Build history of the part. All positions in model axes, mm. A direction names the side the tool comes from. Round coordinates to 2 decimals unless told otherwise and drop trailing zeros. Write each loop counter-clockwise with the first axis right and the second up, starting at its lowest first coordinate (ties: lowest second). Pieces come first, ordered by that corner, then holes.
from build123d import *

# Parameters (mm, degrees)
BOSS_EXTRUDE1_DEPTH = 6
CUT_EXTRUDE1_REACH  = 68.303
SKETCH2_R           = 4.5
CHAMFER1_SIZE       = 10


with BuildPart() as part:
    # Sketch1 → Boss-Extrude1 (new body)
    with BuildSketch(Plane.XY):
        Polygon((-33.521587555, -18.6224812), (-33.521587555, 51.3775188), (-3.521587555, 51.3775188), (-3.521587555, 23.144505274), (41.478412445, 23.144505274), (41.478412445, -18.6224812), align=None)
    extrude(amount=BOSS_EXTRUDE1_DEPTH)

    # Sketch2 → Cut-Extrude1 (cut, up to next)
    with BuildSketch(Plane.XY.offset(6), mode=Mode.PRIVATE) as cut_extrude1_sk1:
        with Locations((-18.521587555, 36.3775188)):
            Circle(SKETCH2_R)
    cut_extrude1_tool1 = extrude(cut_extrude1_sk1.sketch, amount=-CUT_EXTRUDE1_REACH, mode=Mode.PRIVATE) & part.part
    add(cut_extrude1_tool1.solids().sort_by_distance((-18.521588, 36.377519, 6))[0], mode=Mode.SUBTRACT)

    # Chamfer1
    chamfer1_edges = [part.edges().sort_by_distance(p)[0] for p in [
        (-33.521587555, -18.6224812, 3),
    ]]
    chamfer(chamfer1_edges, length=CHAMFER1_SIZE)


solid = part.part
1) Which spindle directions (+Z, -Z, +X, -X, +Y, -Y) get a long thin tool onto all of the face, cutting with end or side? Do faces 1 (the flat face through (-3.522, 37, 3)), 2 (the flat face through (-4, 9, 6)). Say none if no direction does.
Results:
face 1: +Z, -Z, +X, +Y
face 2: +Z, +X, -X, +Y, -Y
2) Mould opens along Y. For faces 3 (the flat face through (-28.452, -13.692, 2.958)), 4 (the cylindrical face through (-19.497, 31.985, 3.042)), 5 (the flat face through (-19, 51.378, 3)) say: released by +Y, released by -Y, zero draft, split by the parting line, or undercut.
Results:
face 3: released by -Y
face 4: undercut
face 5: released by +Y
3) Pin check, flat tip, straight feed: pin 1 Ø1.8 at (y, z) = (31, 1.5) entering from +X. Stop position of the tip, or through.
Results:
pin 1: stops at x = -3.52
4) Slice it at A-A (x = -17). Write the cut outline in (y, z).
Results:
outline: (-18.62, 0) - (32.14, 0) - (32.14, 6) - (-18.62, 6) - close; (40.61, 0) - (51.38, 0) - (51.38, 6) - (40.61, 6) - close
5) Wall check: L1, parallel to Y at x = 17.5, z = 3.35; L2, parallel to Y at x = -22.5, z = 1.2; L3, parallel to Y at x = -20.5, z = 3.75. Give the ranges that are in metal, low to high.
Results:
L1: y = -18.62 to 23.14
L2: y = -18.62 to 34.27, 38.48 to 51.38
L3: y = -18.62 to 32.34, 40.42 to 51.38
6) Slice it at B-B (z = 2.8). Write the cut outline in (x, y).
Results:
outline: (-33.52, -8.62) - (-23.52, -18.62) - (41.48, -18.62) - (41.48, 23.14) - (-3.52, 23.14) - (-3.52, 51.38) - (-33.52, 51.38) - close; hole circle Ø9 at (-18.52, 36.38)
7) Slice it at C-C (y = 28). Write the cut outline in (x, z).
Results:
outline: (-33.52, 0) - (-3.52, 0) - (-3.52, 6) - (-33.52, 6) - close
8) Slice it at D-D (x = 34). Write the cut outline in (y, z).
Results:
outline: (-18.62, 0) - (23.14, 0) - (23.14, 6) - (-18.62, 6) - close
